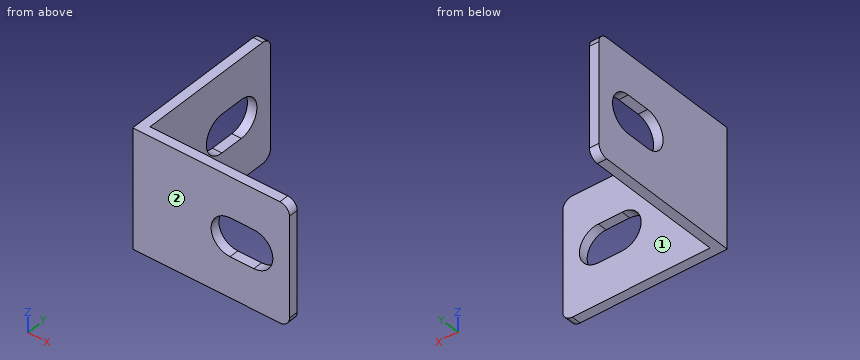
```python
from build123d import *

# Parameters (mm, degrees)
EXTRUDE_1_DEPTH     = 25
FILLET_1_R          = 2
CUT_EXTRUDE_1_DEPTH = 52.720402164
CUT_EXTRUDE_2_DEPTH = 52.720402164


with BuildPart() as part:
    # 草图1 → 凸台-拉伸1 (new body)
    with BuildSketch(Plane.XY):
        Polygon((0, 0), (33, 0), (33, 2), (2, 2), (2, 33), (0, 33), align=None)
    extrude(amount=EXTRUDE_1_DEPTH)

    # 圆角1
    fillet_1_edges = [part.edges().sort_by_distance(p)[0] for p in [
        (33, 1, 25),
        (1, 33, 25),
        (1, 33, 0),
        (33, 1, 0),
    ]]
    fillet(fillet_1_edges, radius=FILLET_1_R)

    # 草图2 → 切除-拉伸1 (cut, through all)
    with BuildSketch(Plane(origin=(0, 2, 0), x_dir=(1, 0, 0), z_dir=(0, 1, 0))):
        with BuildLine():
            Line((20.5, -8.5), (25.5, -8.5))
            ThreePointArc((25.5, -8.5), (29.5, -12.5), (25.5, -16.5))
            Line((25.5, -16.5), (20.5, -16.5))
            ThreePointArc((20.5, -16.5), (16.5, -12.5), (20.5, -8.5))
        make_face()
    extrude(amount=-CUT_EXTRUDE_1_DEPTH, mode=Mode.SUBTRACT)

    # 草图4 → 切除-拉伸2 (cut, through all)
    with BuildSketch(Plane(origin=(2, 0, 0), x_dir=(0, 0, -1), z_dir=(1, 0, 0))):
        with BuildLine():
            Line((-8.5, 25.5), (-8.5, 20.5))
            ThreePointArc((-8.5, 20.5), (-12.5, 16.5), (-16.5, 20.5))
            Line((-16.5, 20.5), (-16.5, 25.5))
            ThreePointArc((-16.5, 25.5), (-12.5, 29.5), (-8.5, 25.5))
        make_face()
    extrude(amount=-CUT_EXTRUDE_2_DEPTH, mode=Mode.SUBTRACT)


solid = part.part
```
The model under review builds one solid part; all positions refer to its coordinate system, in mm. Face numbers are marked on the shaded views. A direction names the side the tool comes from. Round coordinates to 2 decimals unless told otherwise and drop trailing zeros. Order: outer loops, then holes, each group sorted by start corner. A loop starts at its lowest first (then second) coordinate and runs counter-clockwise, first axis right, second up.
(1) For P1, Ø12, axis at x = 21.5, z = 10.5, coming from the +Y side; P2, Ø10, axis at y = 29, z = 5, coming from the -X side, all flat-tipped, find the tip position at first contact; note any pin that passes through.
Working result:
P1: stops at y = 2
P2: stops at x = 0
(2) Take a section at D-D, the plane z = 15.5. State the section outline as (x, y) points.
Working result:
outline: (0, 0) - (17.85, 0) - (17.85, 2) - (2, 2) - (2, 17.85) - (0, 17.85) - close; (0, 28.15) - (2, 28.15) - (2, 33) - (0, 33) - close; (28.15, 0) - (33, 0) - (33, 2) - (28.15, 2) - close
(3) Tool access review of the marked faces 1 and 2: name each direction out of +Z, -Z, +X, -X, +Y, -Y from which nothing blocks a thin tool from reaching the whole face with its end or side.
Working result:
face 1: +Z, -Z, +X, +Y
face 2: +Z, -Z, +X, -X, -Y
(4) Take a section at A-A, the plane y = 24. State the section outline as (x, z) points.
Working result:
outline: (0, 0) - (2, 0) - (2, 8.5) - (0, 8.5) - close; (0, 16.5) - (2, 16.5) - (2, 25) - (0, 25) - close
(5) Take a section at C-C, the plane z = 12.5. State the section outline as (x, y) points, plus the area to 3 significant figures.
Working result:
outline: (0, 0) - (16.5, 0) - (16.5, 2) - (2, 2) - (2, 16.5) - (0, 16.5) - close; (0, 29.5) - (2, 29.5) - (2, 33) - (0, 33) - close; (29.5, 0) - (33, 0) - (33, 2) - (29.5, 2) - close
area: 76.0 mm2
(6) Wall thickness on L1, parallel to Y at x = 12, z = 21: over which ranges is the line inside the solid? List them lowest first.
Working result:
L1: y = 0 to 2
